```python
from build123d import *


with BuildPart() as part:
    # Sketch2 → Revolve1 (revolve)
    with BuildSketch(Plane.XY):
        Polygon((-8.5, 14), (-8.5, -0.10996164), (-8, -0.10996164), (-5.101647841, 3.344159959), (-5.101647841, 4.665808374), (-6.5, 4.665808374), (-6.5, 13), (0, 13), (0, 14), align=None)
    revolve(axis=Axis((0, 14, 0), (0, -1, 0)))


solid = part.part
```
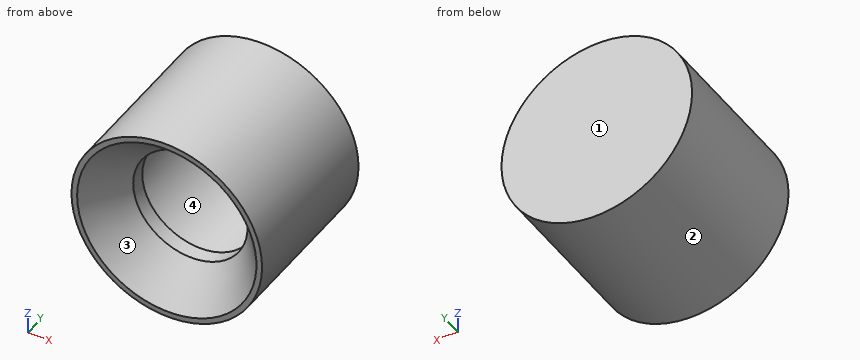
Here's how the part is built. I have some questions about the finished solid (model axes, mm). Face numbers are marked on the shaded views. Give positions to 0.01 mm unless a question says otherwise; leave off trailing zeros. Loops run counter-clockwise (first coordinate to the right, second up) from the corner with the lowest first, then second, coordinate; pieces in that order, holes last. Notation, with made-up numbers: M 36,62.25 L 62,62.25 A22 ccw 62,77.25 Z; hole C -4.75,32 d2. An arc over 180 degrees is marked long. Return JSON: item names as keys, results as strings.
Item 1: Thinking about a two-plate mould opening in Z: for the marked faces 1, 2, 3 and 4, which applies, released by +Z, released by -Z, zero draft, split by the parting line, or undercut?
A:
{"face 1": "zero draft", "face 2": "split by the parting line", "face 3": "undercut", "face 4": "undercut"}
Item 2: Imagine slicing it at D-D on y = 2.75. List the corners of the cut face in (x, z) for me, then the cut area to 3 significant figures.
A:
{"outline": "C 0,0 d17; hole C 0,0 d11.2", "area": "128 mm^2"}
Item 3: Imagine slicing it at B-B on z = 0. List the corners of the cut face in (x, y) for me, then the cut area to 3 significant figures.
A:
{"outline": "M -8.5,-0.11 L -8,-0.11 L -5.1,3.34 L -5.1,4.67 L -6.5,4.67 L -6.5,13 L 6.5,13 L 6.5,4.67 L 5.1,4.67 L 5.1,3.34 L 8,-0.11 L 8.5,-0.11 L 8.5,14 L -8.5,14 Z", "area": "72.8 mm^2"}
Item 4: I'm going to push flat-ended pins straight in: pin 1 Ø6 at (x, y) = (6.5, 7.5) entering from -Z; pin 2 Ø3 at (y, z) = (3.5, -6) entering from +X; pin 3 Ø2 at (y, z) = (7.5, -1.5) entering from -X. Where does each tip first touch, or does it pass through?
A:
{"pin 1": "stops at z = -7.75", "pin 2": "stops at x = 7.21", "pin 3": "stops at x = -8.49"}
Item 5: Imagine slicing it at C-C on y = 7.25. List the corners of the cut face in (x, z) for me, then the cut area to 3 significant figures.
A:
{"outline": "C 0,0 d17; hole C 0,0 d13", "area": "94.2 mm^2"}
Item 6: Please list where these lines run through material, in increasing order: line 1 (X direction, y = 10.5, z = 0); line 2 (X direction, y = 4.2, z = 0).
A:
{"line 1": "x = -8.5 to -6.5, 6.5 to 8.5", "line 2": "x = -8.5 to -5.1, 5.1 to 8.5"}
Item 7: Imagine slicing it at A-A on x = 0. List the corners of the cut face in (y, z) for me.
A:
{"outline": "M -0.11,-8.5 L 14,-8.5 L 14,8.5 L -0.11,8.5 L -0.11,8 L 3.34,5.1 L 4.67,5.1 L 4.67,6.5 L 13,6.5 L 13,-6.5 L 4.67,-6.5 L 4.67,-5.1 L 3.34,-5.1 L -0.11,-8 Z"}
